For this review, use the dimensioned drawing (mm, ordinates from the lowest corner) and the shaded views. A direction names the side the tool comes from. Coordinates: 2 decimals unless noted, no trailing zeros. Loops run counter-clockwise (first coordinate to the right, second up) from the corner with the lowest first, then second, coordinate; pieces in that order, holes last. Notation, with made-up numbers: M 76.25,33 L 127.25,33 A29 cw 127.25,64 Z; hole C 47.5,52 d6. An arc over 180 degrees is marked long. Write item = value, one per line.
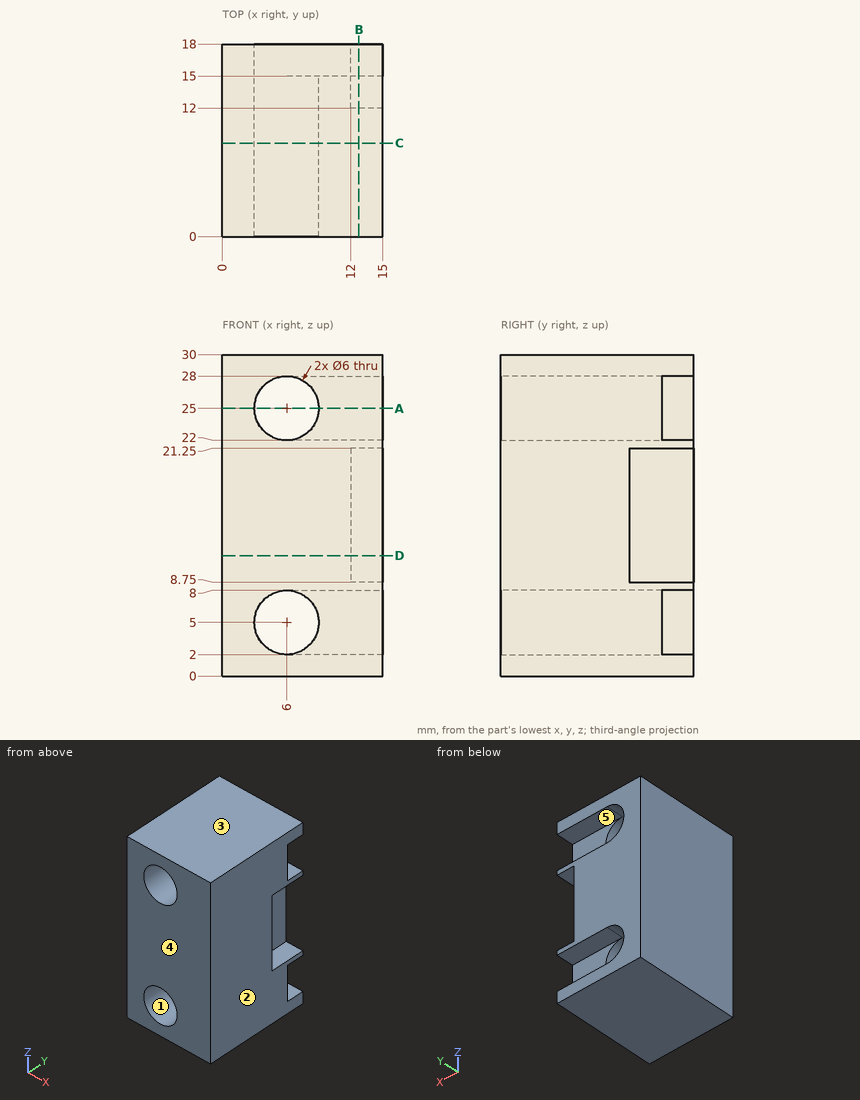
Q1. Machinability: for the marked faces 4 and 5, which of the approach directions +Z, -Z, +X, -X, +Y, -Y give a long, thin tool a straight path to every point of the face, cutting with its end or side? Answer none if there is none.
Solved:
face_4 = +Z, -Z, +X, -X, -Y
face_5 = +X, +Y
Q2. For pin 1 Ø3.5 at (x, y) = (9, 16) entering from -Z; pin 2 Ø1.8 at (x, z) = (9, 24.5) entering from +Y; pin 3 Ø0.9 at (x, z) = (14, 16) entering from +Y; pin 4 Ø3.5 at (x, z) = (6, 25) entering from -Y, all flat-tipped, find the tip position at first contact; note any pin that passes through.
Solved:
pin_1 = 0
pin_2 = 15
pin_3 = 12
pin_4 = through
Q3. Draft analysis for pull direction Z (two halves, no side actions). For the marked faces 1, 2 and 3, state which applies: +Z half, -Z half, draft (parallel to the pull), parting line (faces both ways), or undercut.
Solved:
face_1 = undercut
face_2 = draft
face_3 = +Z half
Q4. Add section A-A (z = 25). Write out the cut boundary in (x, y), and give its area (3 significant figures).
Solved:
outline = M 0,0 L 3,0 L 3,18 L 0,18 Z; M 9,0 L 15,0 L 15,15 L 9,15 Z
area = 144 mm²
Q5. Add section C-C (y = 8.75). Write out the cut boundary in (x, z), and give its area (3 significant figures).
Solved:
outline = M 0,0 L 15,0 L 15,30 L 0,30 Z; hole C 6,5 d6; hole C 6,25 d6
area = 393 mm²
Q6. Add section D-D (z = 11.25). Write out the cut boundary in (x, y), and give its area (3 significant figures).
Solved:
outline = M 0,0 L 15,0 L 15,12 L 12,12 L 12,18 L 0,18 Z
area = 252 mm²
Q7. Add section B-B (x = 12.75). Write out the cut boundary in (y, z).
Solved:
outline = M 0,0 L 18,0 L 18,2 L 15,2 L 15,8 L 18,8 L 18,8.75 L 12,8.75 L 12,21.25 L 18,21.25 L 18,22 L 15,22 L 15,28 L 18,28 L 18,30 L 0,30 Z
Q8. For line 1 along Z through (x, y) = (6, 9); line 2 along X through (y, z) = (7, 25); line 3 along Z through (x, y) = (12.5, 14.5), list the stretches that pass through material, from the lowest coordinate up.
Solved:
line_1 = 0 to 2, 8 to 22, 28 to 30
line_2 = 0 to 3, 9 to 15
line_3 = 0 to 8.75, 21.25 to 30
